from build123d import *

# Parameters (mm, degrees)
SKETCH1_W               = 50
SKETCH1_H               = 10
BOSS_EXTRUDE1_DEPTH     = 10
SKETCH2_R               = 3
CUT_EXTRUDE1_DEPTH      = 10
SKETCH3_R               = 2
CUT_EXTRUDE2_DEPTH      = 10
BOSS_EXTRUDE2_DEPTH     = 30
CUT_EXTRUDE4_DEPTH      = 61.464865831
CUT_EXTRUDE4_DEPTH_BACK = 61.464865831
SKETCH6_W               = 47
SKETCH6_H               = 25
CUT_EXTRUDE5_DEPTH      = 54.150729064
CUT_EXTRUDE5_DEPTH_BACK = 54.150729064
SKETCH7_R               = 2
SKETCH5_R               = 6.5
CUT_EXTRUDE6_DEPTH      = 66.76473219


with BuildPart() as part:
    # Sketch1 → Boss-Extrude1 (new body)
    with BuildSketch(Plane(origin=(0, 0, 0), x_dir=(1, 0, 0), z_dir=(0, 1, 0))):
        with Locations((25, -5)):
            Rectangle(SKETCH1_W, SKETCH1_H)
    extrude(amount=BOSS_EXTRUDE1_DEPTH)

    # Sketch2 → Cut-Extrude1 (cut)
    with BuildSketch(Plane(origin=(0, 10, 0), x_dir=(1, 0, 0), z_dir=(0, 1, 0))):
        with Locations(Location((23, -5, 0), (0, 0, 270))):
            Circle(SKETCH2_R)
    extrude(amount=-CUT_EXTRUDE1_DEPTH, mode=Mode.SUBTRACT)

    # Sketch3 → Cut-Extrude2 (cut)
    with BuildSketch(Plane.XY.offset(10)):
        with Locations((8, 5)):
            Circle(SKETCH3_R)
        with Locations((16, 5)):
            Circle(SKETCH3_R)
        with Locations(Location((42, 5, 0), (0, 0, 180))):
            Circle(SKETCH3_R)
        with Locations(Location((34, 5, 0), (0, 0, 180))):
            Circle(SKETCH3_R)
    extrude(amount=-CUT_EXTRUDE2_DEPTH, mode=Mode.SUBTRACT)

    # Sketch4 → Boss-Extrude2 (add)
    with BuildSketch(Plane(origin=(0, 0, 0), x_dir=(-1, 0, 0), z_dir=(0, 0, -1))):
        with BuildLine():
            Line((-16, 11), (-4, 11))
            ThreePointArc((-4, 11), (14, 5), (-4, -1))
            Line((-4, -1), (-16, -1))
            ThreePointArc((-16, -1), (-22, 5), (-16, 11))
        make_face()
    extrude(amount=BOSS_EXTRUDE2_DEPTH)

    # Sketch6 → Cut-Extrude4 (cut, two sides: drawn at the far end of the back side and taken through both)
    with BuildSketch(Plane.XZ.offset(1).offset(-CUT_EXTRUDE4_DEPTH_BACK)):
        with Locations((4.191332745, -20.5)):
            Rectangle(SKETCH6_W, SKETCH6_H)
    extrude(amount=CUT_EXTRUDE4_DEPTH + CUT_EXTRUDE4_DEPTH_BACK, mode=Mode.SUBTRACT)

    # Sketch7 → Cut-Extrude5 (cut, two sides: drawn at the far end of the back side and taken through both)
    with BuildSketch(Plane.XY.offset(-CUT_EXTRUDE5_DEPTH_BACK)):
        with Locations((8, 5)):
            Circle(SKETCH7_R)
        with Locations((16, 5)):
            Circle(SKETCH7_R)
    extrude(amount=CUT_EXTRUDE5_DEPTH + CUT_EXTRUDE5_DEPTH_BACK, mode=Mode.SUBTRACT)

    # Sketch5 → Cut-Extrude6 (cut, through all)
    with BuildSketch(Plane(origin=(0, 0, -30), x_dir=(-1, 0, 0), z_dir=(0, 0, -1))):
        with Locations(Location((4, 5, 0), (0, 0, 230.284862768))):
            Circle(SKETCH5_R)
    extrude(amount=-CUT_EXTRUDE6_DEPTH, mode=Mode.SUBTRACT)


solid = part.part
For this review, take the finished solid that the model builds, in its own axes (mm). A direction names the side the tool comes from. Give positions to 0.01 mm unless a question says otherwise; leave off trailing zeros. Loops run counter-clockwise (first coordinate to the right, second up) from the corner with the lowest first, then second, coordinate; pieces in that order, holes last. Notation, with made-up numbers: (43, 44.5) -> (99, 44.5) arc R31 ccw to (99, 72.5) -> close; hole circle Ø3 at (-29, -17). An arc over 180 degrees is marked (long way). One line per question, with ' | ' between items.
1) Insertion check: pin 1 Ø8 at (x, z) = (17, 5.5) entering from -Y; pin 2 Ø2.5 at (x, z) = (8, -2.5) entering from +Y; pin 3 Ø1 at (x, y) = (38, -1) entering from -Z; pin 4 Ø10 at (x, z) = (10, 6.5) entering from +Y. Each pin has a flat end and moves straight along its axis. Give the tip position at first contact, or say it passes through.
Resolved:
pin 1: stops at y = 0 | pin 2: stops at y = 11 | pin 3: passes through | pin 4: stops at y = 10
2) We need section D-D (x = 34). Write out the cut boundary in (y, z).
Resolved:
outline: (0, 0) -> (3, 0) -> (3, 10) -> (0, 10) -> close; (7, 0) -> (10, 0) -> (10, 10) -> (7, 10) -> close
3) We need section B-B (x = -4). Write out the cut boundary in (y, z), plus the area to 3 significant figures.
Resolved:
outline: (-5, -8) -> (-1.5, -8) -> (-1.5, 0) -> (-5, 0) -> close; (11.5, -8) -> (15, -8) -> (15, 0) -> (11.5, 0) -> close | area: 56.0 mm2
4) The part is to be moulded in two halves that separate along Y. For faces 1 (the cylindrical face through (32.153, 5.766, 5.07)), 2 (the cylindrical face through (22, 5, -4)), 3 (the cylindrical face through (44, 5, 5)), 4 (the flat face through (4, 5, -8)), say which applies: +Y half, -Y half, draft (parallel to the pull), parting line (faces both ways), or undercut.
Resolved:
face 1: undercut | face 2: parting line | face 3: undercut | face 4: draft
5) For faces 5 (the flat face through (10, 11, -4)), 6 (the flat face through (25, 10, 2)), 7 (the flat face through (10, -1, -4)), list the 3-axis set-ups (+Z, -Z, +X, -X, +Y, -Y) from which the entire face can be reached by the end or side of a thin tool; tool diameter is ignored.
Resolved:
face 5: +Z, -Z, +X, +Y | face 6: +Z, +X, -X, +Y | face 7: +Z, -Z, +X, -Y
6) We need section C-C (y = 1.25). Write out the cut boundary in (x, z), plus the area to 3 significant figures.
Resolved:
outline: (-13.27, -8) -> (-9.31, -8) -> (-9.31, 0) -> (-13.27, 0) -> close; (1.31, -8) -> (20.68, -8) -> (20.68, 0) -> (50, 0) -> (50, 10) -> (1.31, 10) -> close; hole circle Ø6 at (23, 5) | area: 645 mm2
7) We need section A-A (z = 5). Write out the cut boundary in (x, y), plus the area to 3 significant figures.
Resolved:
outline: (0.15, 0) -> (20, 0) -> (20, 10) -> (0.15, 10) arc R6.5 cw to start; (26, 0) -> (50, 0) -> (50, 10) -> (26, 10) -> close; hole circle Ø4 at (8, 5); hole circle Ø4 at (16, 5); hole circle Ø4 at (34, 5); hole circle Ø4 at (42, 5) | area: 372 mm2
8) To check wall thickness, follow probe 1 along X at (y, z) = (5, 4.75); probe 2 along X at (y, z) = (5, -1.5); probe 3 along Y at (x, z) = (-4, -3.5). State the ranges of each line that lie inside material, in increasing order.
Resolved:
probe 1: x = 2.5 to 6, 10 to 14, 18 to 20.01, 25.99 to 32, 36 to 40, 44 to 50 | probe 2: x = -14 to -10.5, 2.5 to 6, 10 to 14, 18 to 22 | probe 3: y = -5 to -1.5, 11.5 to 15
